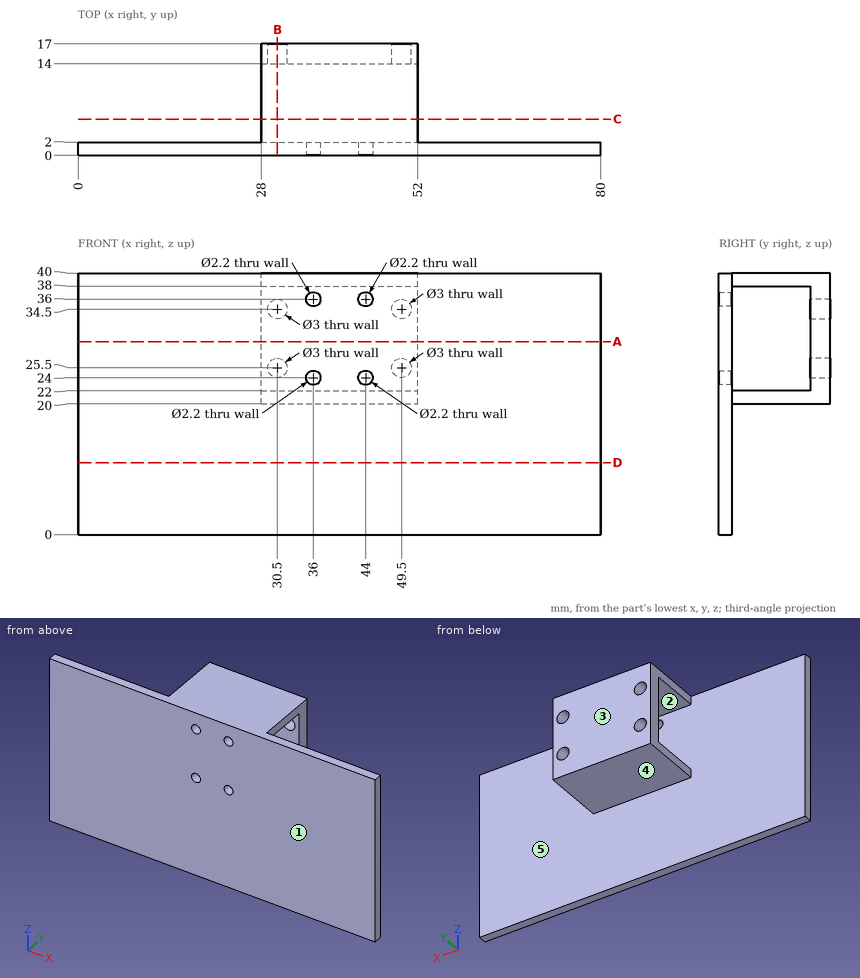
Geometry: see drawing. Coordinates: mm, zero at the bounding-box minimum. A direction names the side the tool comes from. Give positions to 0.01 mm unless a question says otherwise; leave off trailing zeros. Order: outer loops, then holes, each group sorted by start corner. A loop starts at its lowest first (then second) coordinate and runs counter-clockwise, first axis right, second up. Notation, with made-up numbers: M 36,7.25 L 45,7.25 A20 ccw 45,44.25 Z; hole C -21,43.25 d8. An arc over 180 degrees is marked long. Answer as CSV lines item,"result". Start each with the question number.
1) Mould query, pull axis Z, two halves, no side actions, for the marked faces 3, 4 and 5. Classes: +Z half, -Z half, draft (parallel to the pull), parting line (faces both ways), or undercut.
2) Cut plane A-A (z = 29.5). Output: boundary loops of the cut face in (x, y).
3) Cut plane C-C (y = 5.5). Output: boundary loops of the cut face in (x, z), then the cut area to 3 significant figures.
4) Line query: line 1 (X direction, y = 14.95, z = 34.5); line 2 (Y direction, x = 41, z = 30); line 3 (X direction, y = 0.85, z = 24). Output: solid intervals per line, ascending. Write a range as from..to.
5) Cut plane B-B (x = 30.5). Output: boundary loops of the cut face in (y, z).
6) First-contact query: P1, Ø8, axis at y = 11.5, z = 23.5, coming from the -X side; P2, Ø2, axis at x = 9.5, z = 18, coming from the +Y side; P3, Ø10, axis at x = 26.5, y = 12, coming from the -Z side; P4, Ø5, axis at x = 61, y = 6, coming from the +Z side. Flat tips, straight axial feed; report the tip coordinate or a pass-through.
7) Set-up query: the marked faces 1 and 2. Return all of +Z, -Z, +X, -X, +Y, -Y with unobstructed straight access to the full face (end or side cutting, diameter ignored); none if empty.
8) Cut plane D-D (z = 11). Output: boundary loops of the cut face in (x, y), then the cut area to 3 significant figures.
Findings below:
1,face 3,"draft"
1,face 4,"-Z half"
1,face 5,"undercut"
2,outline,"M 0,0 L 80,0 L 80,2 L 0,2 Z; M 28,14 L 52,14 L 52,17 L 28,17 Z"
3,outline,"M 28,20 L 52,20 L 52,22 L 28,22 Z; M 28,38 L 52,38 L 52,40 L 28,40 Z"
3,area,"96.0 mm²"
4,line 1,"x = 28..29, 32..48, 51..52"
4,line 2,"y = 0..2, 14..17"
4,line 3,"x = 0..34.9, 37.1..42.9, 45.1..80"
5,outline,"M 0,0 L 2,0 L 2,20 L 17,20 L 17,24 L 14,24 L 14,22 L 2,22 L 2,38 L 14,38 L 14,36 L 17,36 L 17,40 L 0,40 Z; M 14,27 L 17,27 L 17,33 L 14,33 Z"
6,P1,"stops at x = 28"
6,P2,"stops at y = 2"
6,P3,"stops at z = 20"
6,P4,"passes through"
7,face 1,"+Z, -Z, +X, -X, -Y"
7,face 2,"+X, -X"
8,outline,"M 0,0 L 80,0 L 80,2 L 0,2 Z"
8,area,"160 mm²"
